Source: CAD feature listing. Evaluate the final solid. Frame: model axes, mm. Face numbers are marked on the shaded views. A direction names the side the tool comes from. Give positions to 0.01 mm unless a question says otherwise; leave off trailing zeros. Order: outer loops, then holes, each group sorted by start corner. A loop starts at its lowest first (then second) coordinate and runs counter-clockwise, first axis right, second up. Notation, with made-up numbers: M 43.25,57.25 L 89.25,57.25 A16 ccw 89.25,75.25 Z; hole C 45.25,4 d8. An arc over 180 degrees is marked long. Answer in a Markdown table with one row per item. Add a question column.
(1) Set-up query: the marked faces 5, 6 and 7. Return all of +Z, -Z, +X, -X, +Y, -Y with unobstructed straight access to the full face (end or side cutting, diameter ignored); none if empty.
(2) Section query B-B, the plane y = -2. Return loops of the section in (x, z), plus the area to 3 significant figures.
(3) Section query C-C, the plane z = -29. Return loops of the section in (x, y).
(4) Pin query (flat end, axial travel): P1, Ø5, axis at y = 1.5, z = -18, coming from the -X side; P2, Ø11, axis at x = -56, z = -1.5, coming from the -Y side; P3, Ø19, axis at x = 0, y = 0, coming from the +Z side; P4, Ø2, axis at y = -11.5, z = 2, coming from the -X side. Return the tip coordinate at first contact, or that it passes through.
(5) Section query D-D, the plane y = -20.5. Return loops of the section in (x, z), plus the area to 3 significant figures.
(6) Mould query, pull axis Y, two halves, no side actions, for the marked faces 1, 2, 3 and 4. Classes: pulls with the +Y half, pulls with the -Y half, needs draft (parallel to the pull), parting line crosses it, or undercut.
(7) Material intervals for line 1 along Y through (x, z) = (44, -1); line 2 along Z through (x, y) = (-52, 11); line 3 along Y through (x, z) = (19, 0.5), sorted ascending.
(8) Section query A-A, the plane x = 44. Return loops of the section in (y, z).
from build123d import *

# Parameters (mm, degrees)
BRACKET_PLATE_PROFILE_R  = 6
BRACKET_PLATE_12MM_DEPTH = 6
HUB_AND_BORE_CIRCLES_R   = 16
BORE_32_DEPTH            = 12
HUB_50_DEPTH             = 6
HUB_50_DEPTH_BACK        = 44
SKETCH2_3_R              = 25
SKETCH2_3_R_2            = 16
HUB_SLOT_CUT_DEPTH       = 85.787970845


with BuildPart() as part:
    # Bracket Plate Profile → Bracket Plate 12mm (new, symmetric)
    with BuildSketch(Plane.XY):
        with BuildLine():
            Line((12.75, 30.437435832), (50.181818182, 14.757544646))
            ThreePointArc((50.181818182, 14.757544646), (60, 0), (50.181818182, -14.757544646))
            Line((50.181818182, -14.757544646), (12.75, -30.437435832))
            ThreePointArc((12.75, -30.437435832), (0, -33), (-12.75, -30.437435832))
            Line((-12.75, -30.437435832), (-50.181818182, -14.757544646))
            ThreePointArc((-50.181818182, -14.757544646), (-60, 0), (-50.181818182, 14.757544646))
            Line((-50.181818182, 14.757544646), (-12.75, 30.437435832))
            ThreePointArc((-12.75, 30.437435832), (0, 33), (12.75, 30.437435832))
        make_face()
        with Locations((-44, 0)):
            Circle(BRACKET_PLATE_PROFILE_R, mode=Mode.SUBTRACT)
        with Locations((44, 0)):
            Circle(BRACKET_PLATE_PROFILE_R, mode=Mode.SUBTRACT)
    extrude(amount=BRACKET_PLATE_12MM_DEPTH, both=True)

    # Hub and Bore Circles → Bore _32 (cut)
    with BuildSketch(Plane.XY.offset(6)):
        Circle(HUB_AND_BORE_CIRCLES_R)
    extrude(amount=-BORE_32_DEPTH, mode=Mode.SUBTRACT)

    # Sketch2_3 → Hub _50 (add, two sides: drawn at the far end of the back side and taken through both)
    with BuildSketch(Plane.XY.offset(6).offset(-HUB_50_DEPTH_BACK)):
        Circle(SKETCH2_3_R)
        Circle(SKETCH2_3_R_2, mode=Mode.SUBTRACT)
    extrude(amount=HUB_50_DEPTH + HUB_50_DEPTH_BACK)

    # Hub Slot Profile → Hub Slot Cut (cut, through all)
    with BuildSketch(Plane(origin=(0, 0, -38), x_dir=(-1, 0, 0), z_dir=(0, 0, -1))):
        Polygon((0, 0), (0, -33), (0, -48.621178417), (74.791991636, 0), (30.829460929, 0), align=None)
    extrude(amount=-HUB_SLOT_CUT_DEPTH, mode=Mode.SUBTRACT)


solid = part.part
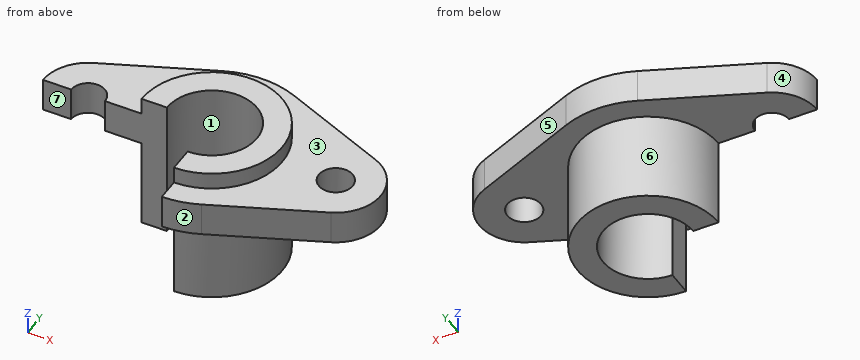
Values follow:
| question | item | result |
|---|---|---|
| 1 | face 5 | +Z, -Z, +X, +Y |
| 1 | face 6 | -Z |
| 1 | face 7 | +Z, -Z, -X, -Y |
| 2 | outline | M 15.87,-38 L 24.92,-38 L 24.92,-6 L 38.34,-6 L 38.34,6 L 24.92,6 L 24.92,12 L 15.87,12 Z; M 49.66,-6 L 59.87,-6 L 59.87,6 L 49.66,6 Z |
| 2 | area | 736 mm² |
| 3 | outline | M -25,0 L -16,0 A16 cw long 0,-16 L 0,-25 A25 ccw long Z |
| 4 | P1 | stops at x = -25 |
| 4 | P2 | stops at y = 0 |
| 4 | P3 | passes through |
| 4 | P4 | stops at x = 9.99 |
| 5 | outline | M 0,-38 L 14.31,-38 L 14.31,-6 L 36.47,-6 L 36.47,6 L 14.31,6 L 14.31,12 L 0,12 Z |
| 5 | area | 981 mm² |
| 6 | face 1 | undercut |
| 6 | face 2 | pulls with the -Y half |
| 6 | face 3 | needs draft |
| 6 | face 4 | pulls with the +Y half |
| 7 | line 1 | y = -17.35 to -6, 6 to 17.35 |
| 7 | line 2 | z = -6 to 6 |
| 7 | line 3 | y = -27.82 to 27.82 |
| 8 | outline | M -17.35,-6 L -6,-6 L -6,6 L -17.35,6 Z; M 6,-6 L 17.35,-6 L 17.35,6 L 6,6 Z |
